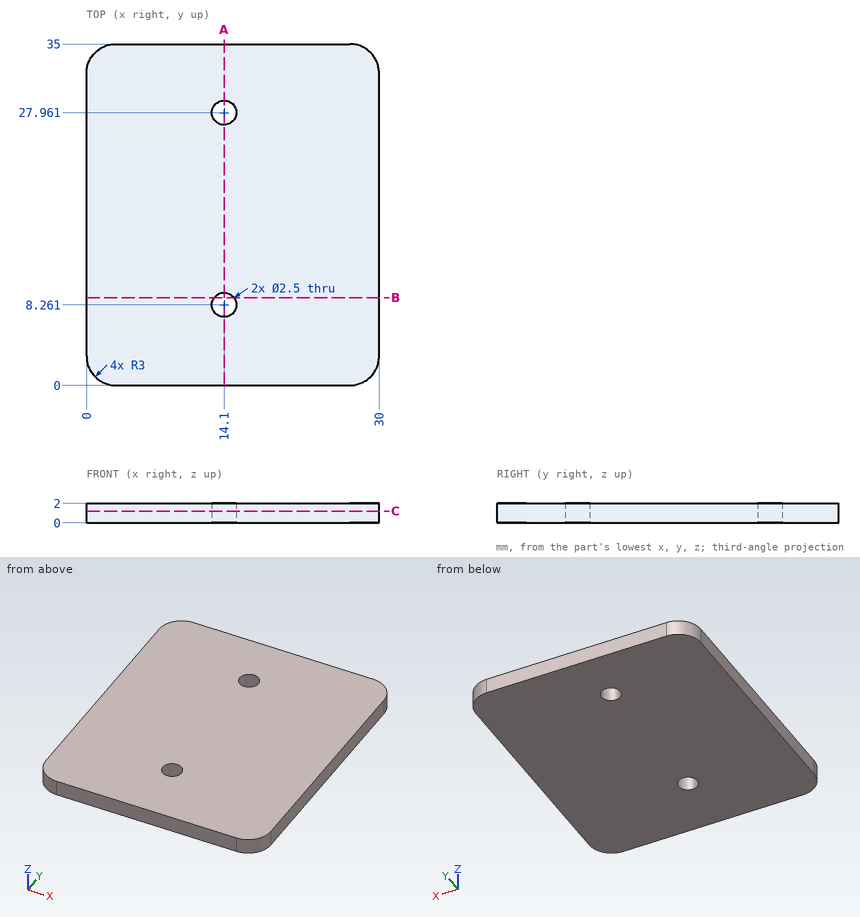
Design review of the part shown in the three views and the two pictorial views. Dimensions are in mm from the part's minimum x, y and z. Coordinates: 2 decimals unless noted, no trailing zeros. Loops run counter-clockwise (first coordinate to the right, second up) from the corner with the lowest first, then second, coordinate; pieces in that order, holes last. Notation, with made-up numbers: (21.25, -38) -> (35.25, -38) arc R31 ccw to (35.25, -5) -> close; hole circle Ø9 at (61.5, -13.75). An arc over 180 degrees is marked (long way). Answer as CSV lines item,"result".
Item 1: Insertion check: pin 1 (2 mm diameter, centred on x = 14.1, y = 8.26, fed in from -Z). The pin has a flat end and moves straight along its axis. Give the tip position at first contact, or say it passes through.
Results below:
pin 1,"passes through"
Item 2: Take a section at C-C, the plane z = 1.2. State the section outline as (x, y) points, and give its area (3 significant figures).
Results below:
outline,"(0, 3) arc R3 ccw to (3, 0) -> (27, 0) arc R3 ccw to (30, 3) -> (30, 32) arc R3 ccw to (27, 35) -> (3, 35) arc R3 ccw to (0, 32) -> close; hole circle Ø2.5 at (14.1, 8.26); hole circle Ø2.5 at (14.1, 27.96)"
area,"1,030 mm2"
Item 3: For L1, parallel to Y at x = 14.1, z = 1.65; L2, parallel to X at y = 7.5, z = 0.75; L3, parallel to X at y = 27, z = 0.15, list the stretches that pass through material, from the lowest coordinate up.
Results below:
L1,"y = 0 to 7.01, 9.51 to 26.71, 29.21 to 35"
L2,"x = 0 to 13.11, 15.09 to 30"
L3,"x = 0 to 13.3, 14.9 to 30"
Item 4: Take a section at B-B, the plane y = 9. State the section outline as (x, z) points.
Results below:
outline,"(0, 0) -> (13.09, 0) -> (13.09, 2) -> (0, 2) -> close; (15.11, 0) -> (30, 0) -> (30, 2) -> (15.11, 2) -> close"
Item 5: Take a section at A-A, the plane x = 14.1. State the section outline as (y, z) points.
Results below:
outline,"(0, 0) -> (7.01, 0) -> (7.01, 2) -> (0, 2) -> close; (9.51, 0) -> (26.71, 0) -> (26.71, 2) -> (9.51, 2) -> close; (29.21, 0) -> (35, 0) -> (35, 2) -> (29.21, 2) -> close"
